Geometry check sheet. Reference: drawing and pictorial views, mm from the part's lowest x, y, z. Give positions to 0.01 mm unless a question says otherwise; leave off trailing zeros. Order: outer loops, then holes, each group sorted by start corner. A loop starts at its lowest first (then second) coordinate and runs counter-clockwise, first axis right, second up.
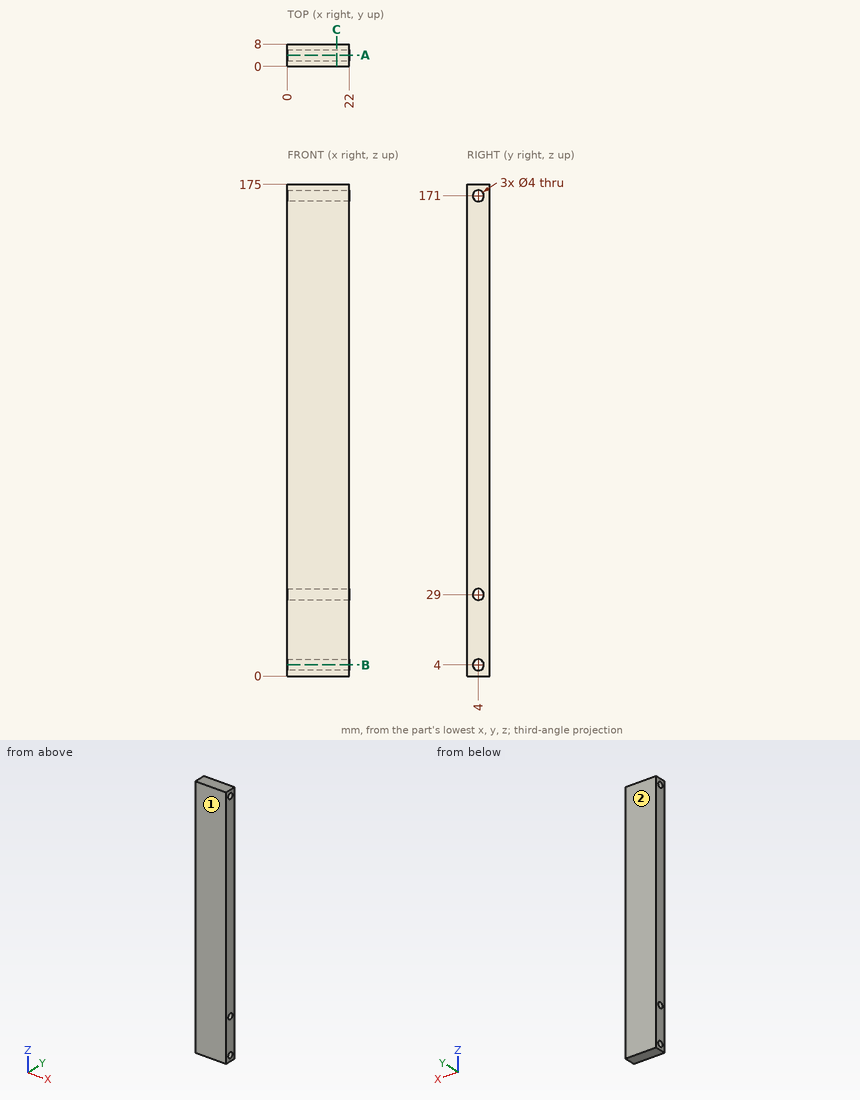
(1) Thickness scan on L1, parallel to Y at x = 6, z = 4; L2, parallel to Z at x = 7, y = 5. Record the ranges inside material, lowest first.
(2) Sectioned sample at C-C (x = 17.5). Enter the section's corners in (y, z), plus the area to 3 significant figures.
(3) Sectioned sample at B-B (z = 4). Enter the section's corners in (x, y), plus the area to 3 significant figures.
(4) Sectioned sample at A-A (y = 4). Enter the section's corners in (x, z), plus the area to 3 significant figures.
(5) Release check for a two-part mould opening along Y. For the marked faces 1 and 2 record: released by +Y, released by -Y, zero draft, split by the parting line, or undercut.
(6) Go/stop test with a flat-tipped pin: P1, Ø3, axis at y = 4, z = 29, coming from the +X side. Record where the tip stops, or that it passes through.
Values follow:
1. L1: y = 0 to 2, 6 to 8
1. L2: z = 0 to 2.27, 5.73 to 27.27, 30.73 to 169.27, 172.73 to 175
2. outline: (0, 0) - (8, 0) - (8, 175) - (0, 175) - close; hole circle Ø4 at (4, 4); hole circle Ø4 at (4, 29); hole circle Ø4 at (4, 171)
2. area: 1,360 mm2
3. outline: (0, 0) - (22, 0) - (22, 2) - (0, 2) - close; (0, 6) - (22, 6) - (22, 8) - (0, 8) - close
3. area: 88.0 mm2
4. outline: (0, 0) - (22, 0) - (22, 2) - (0, 2) - close; (0, 6) - (22, 6) - (22, 27) - (0, 27) - close; (0, 31) - (22, 31) - (22, 169) - (0, 169) - close; (0, 173) - (22, 173) - (22, 175) - (0, 175) - close
4. area: 3,590 mm2
5. face 1: released by -Y
5. face 2: released by +Y
6. P1: passes through
